Geometry: see drawing. Coordinates: mm, zero at the bounding-box minimum. Give positions to 0.01 mm unless a question says otherwise; leave off trailing zeros. Order: outer loops, then holes, each group sorted by start corner. A loop starts at its lowest first (then second) coordinate and runs counter-clockwise, first axis right, second up. Notation, with made-up numbers: M 20,79 L 49,79 A25 ccw 49,96 Z; hole C 56,-9 d7. An arc over 180 degrees is marked long. Use a Markdown table: item, result.
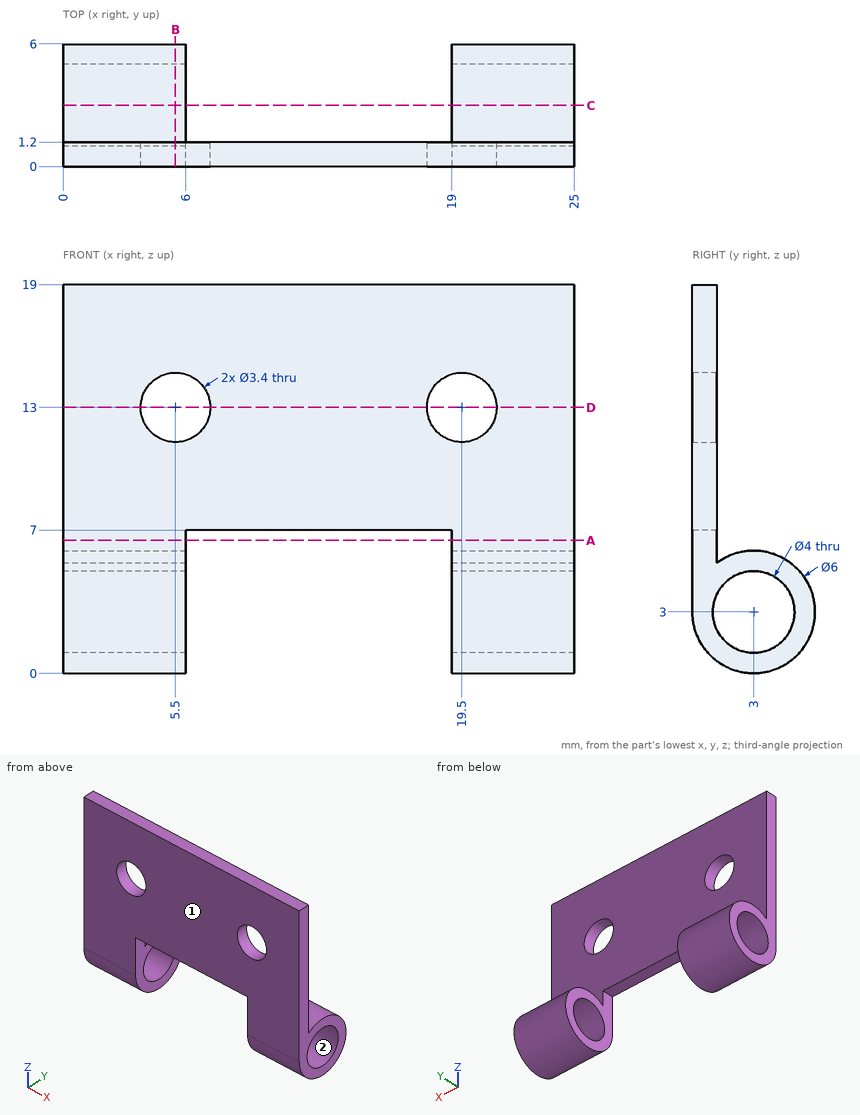
1) Mould query, pull axis Z, two halves, no side actions, for the marked faces 1 and 2. Classes: released by +Z, released by -Z, zero draft, split by the parting line, or undercut.
Response values:
| item | result |
|---|---|
| face 1 | zero draft |
| face 2 | undercut |
2) First-contact query: pin 1 Ø2 at (x, z) = (19.5, 13) entering from -Y; pin 2 Ø0.6 at (x, y) = (13, 0.5) entering from -Z; pin 3 Ø1.5 at (x, z) = (20.5, 8) entering from +Y. Flat tips, straight axial feed; report the tip coordinate or a pass-through.
Response values:
| item | result |
|---|---|
| pin 1 | passes through |
| pin 2 | stops at z = 7 |
| pin 3 | stops at y = 1.2 |
3) Material intervals for line 1 (X direction, y = 0.45, z = 13); line 2 (Z direction, x = 1.3, y = 3), sorted ascending. Write a range as from..to.
Response values:
| item | result |
|---|---|
| line 1 | x = 0..3.8, 7.2..17.8, 21.2..25 |
| line 2 | z = 0..1, 5..6 |
4) Cut plane B-B on x = 5.5. Return loops of the section in (y, z), and give its area (3 significant figures).
Response values:
| item | result |
|---|---|
| outline | M 0,3 A3 ccw long 1.2,5.4 L 1.2,11.3 L 0,11.3 Z; M 0,14.7 L 1.2,14.7 L 1.2,19 L 0,19 Z; hole C 3,3 d4 |
| area | 28.8 mm² |
5) Cut plane A-A on z = 6.5. Return loops of the section in (x, y).
Response values:
| item | result |
|---|---|
| outline | M 0,0 L 6,0 L 6,1.2 L 0,1.2 Z; M 19,0 L 25,0 L 25,1.2 L 19,1.2 Z |
6) Cut plane D-D on z = 13. Return loops of the section in (x, y), and give its area (3 significant figures).
Response values:
| item | result |
|---|---|
| outline | M 0,0 L 3.8,0 L 3.8,1.2 L 0,1.2 Z; M 7.2,0 L 17.8,0 L 17.8,1.2 L 7.2,1.2 Z; M 21.2,0 L 25,0 L 25,1.2 L 21.2,1.2 Z |
| area | 21.8 mm² |
7) Cut plane C-C on y = 3. Return loops of the section in (x, z).
Response values:
| item | result |
|---|---|
| outline | M 0,0 L 6,0 L 6,1 L 0,1 Z; M 0,5 L 6,5 L 6,6 L 0,6 Z; M 19,0 L 25,0 L 25,1 L 19,1 Z; M 19,5 L 25,5 L 25,6 L 19,6 Z |
